Part model, mm, in its own coordinate system. Face numbers are marked on the shaded views. A direction names the side the tool comes from. Give positions to 0.01 mm unless a question says otherwise; leave off trailing zeros. Order: outer loops, then holes, each group sorted by start corner. A loop starts at its lowest first (then second) coordinate and runs counter-clockwise, first axis right, second up. Notation, with made-up numbers: (28, 81) - (77, 81) arc R15 cw to (77, 100) - close; hole circle Ø10 at (61.5, 25). An arc over 180 degrees is marked (long way). One line per item, written item: value.
```python
from build123d import *

# Parameters (mm, degrees)
BOSS_EXTRUDE1_DEPTH = 45
SKETCH4_R           = 25
BOSS_EXTRUDE2_DEPTH = 445
CHAMFER2_SIZE       = 4


with BuildPart() as part:
    # Sketch1 → Boss-Extrude1 (new body)
    with BuildSketch(Plane.XY):
        Polygon((30.022213998, -52), (60.044427996, 0), (30.022213998, 52), (-30.022213998, 52), (-60.044427996, 0), (-30.022213998, -52), align=None)
    extrude(amount=BOSS_EXTRUDE1_DEPTH)

    # Sketch3 → Cut-Revolve3 (revolve, cut)
    with BuildSketch(Plane(origin=(0, 0, 0), x_dir=(1, 0, 0), z_dir=(0, 1, 0))):
        with BuildLine():
            Line((-60.044427996, -12), (-60.044427996, 0))
            Line((-60.044427996, 0), (-48.044427996, 0))
            ThreePointArc((-48.044427996, 0), (-56.52970937, -3.514718626), (-60.044427996, -12))
        make_face()
    revolve(axis=Axis((0, 0, -19.888042613), (0, 0, 1)), mode=Mode.SUBTRACT)

    # Sketch4 → Boss-Extrude2 (add)
    with BuildSketch(Plane.XY.offset(45)):
        Circle(SKETCH4_R)
    extrude(amount=BOSS_EXTRUDE2_DEPTH)

    # Chamfer2
    chamfer2_edges = [part.edges().sort_by_distance(p)[0] for p in [
        (-25, 0, 490),
    ]]
    chamfer(chamfer2_edges, length=CHAMFER2_SIZE)


solid = part.part
```
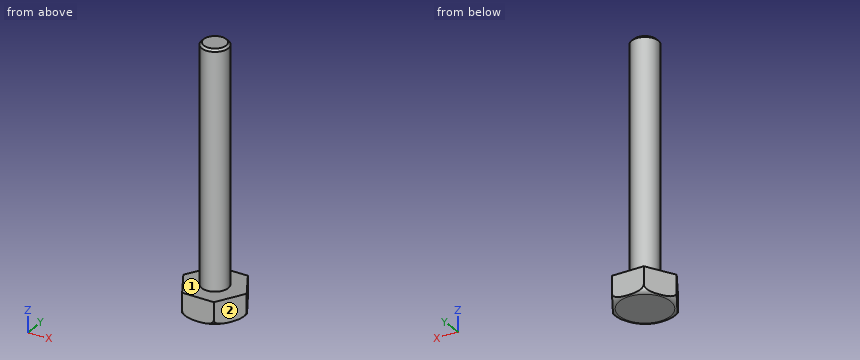
1) Wall check: line 1 along Z through (x, y) = (36.5, -28); line 2 along Z through (x, y) = (-18, -11); line 3 along Y through (x, z) = (15.5, 294.5). Give the ranges that are in metal, low to high. Write a range as [from, to].
Answer:
line 1: z = [0, 45]
line 2: z = [0, 489.9]
line 3: y = [-19.62, 19.62]
2) Drop flat-ended pins along their axis: P1, Ø4, axis at y = 22.5, z = 341, coming from the -X side; P2, Ø5, axis at x = 34.5, y = 36.5, coming from the +Z side. Give the stop position or say it passes through.
Answer:
P1: stops at x = -14.31
P2: stops at z = 45
3) Which spindle directions (+Z, -Z, +X, -X, +Y, -Y) get a long thin tool onto all of the face, cutting with end or side? Do the marked faces 1 and 2. Say none if no direction does.
Answer:
face 1: +Z
face 2: +Z, -Z, +X, -Y
4) Slice it at A-A on x = 0. Write the cut outline in (y, z).
Answer:
outline: (-52, 0.67) arc R12 ccw to (-48.04, 0) - (48.04, 0) arc R12 ccw to (52, 0.67) - (52, 45) - (25, 45) - (25, 486) - (21, 490) - (-21, 490) - (-25, 486) - (-25, 45) - (-52, 45) - close
5) Slice it at B-B on z = 417.5. Write the cut outline in (x, y).
Answer:
outline: circle Ø50 at (0, 0)
